from build123d import *

# Parameters (mm, degrees)
FILLET1_R           = 1
SKETCH2_R           = 10
BOSS_EXTRUDE1_DEPTH = 2.5
CUT_EXTRUDE1_DEPTH  = 10.5
BOSS_EXTRUDE2_DEPTH = 13.5


with BuildPart() as part:
    # Sketch1 → Revolve1 (revolve)
    with BuildSketch(Plane.XY):
        with BuildLine():
            Line((20, 8.32575695), (20, 0))
            Line((20, 0), (0, 0))
            Line((0, 0), (0, 12.5))
            ThreePointArc((0, 12.5), (10.215482184, 11.445315647), (20, 8.32575695))
        make_face()
    revolve(axis=Axis((0, 0, 0), (0, 1, 0)))

    # Fillet1
    fillet1_edges = [part.edges().sort_by_distance(p)[0] for p in [
        (-20, 8.32575695, 0),
    ]]
    fillet(fillet1_edges, radius=FILLET1_R)

    # Sketch2 → Boss-Extrude1 (add)
    with BuildSketch(Plane.XZ):
        Circle(SKETCH2_R)
    extrude(amount=BOSS_EXTRUDE1_DEPTH)

    # Sketch3 → Cut-Extrude1 (cut)
    with BuildSketch(Plane(origin=(0, 8, 0), x_dir=(-1, 0, 0), z_dir=(0, -1, 0))):
        with BuildLine():
            Line((7.5, 8), (7.5, -8))
            ThreePointArc((7.5, -8), (10.299205094, -11.811908762), (14.774238712, -10.282114106))
            ThreePointArc((14.774238712, -10.282114106), (18, 0), (14.774238712, 10.282114106))
            ThreePointArc((14.774238712, 10.282114106), (10.299205094, 11.811908762), (7.5, 8))
        make_face()
        with BuildLine():
            Line((-7.5, 8), (-7.5, -8))
            ThreePointArc((-7.5, -8), (-10.299205094, -11.811908762), (-14.774238712, -10.282114106))
            ThreePointArc((-14.774238712, -10.282114106), (-18, 0), (-14.774238712, 10.282114106))
            ThreePointArc((-14.774238712, 10.282114106), (-10.299205094, 11.811908762), (-7.5, 8))
        make_face()
    extrude(amount=-CUT_EXTRUDE1_DEPTH, mode=Mode.SUBTRACT)

    # Sketch5 → Boss-Extrude2 (add)
    with BuildSketch(Plane.XZ):
        Polygon((2, -12), (0, -15.464101615), (-2, -12), align=None)
        Polygon((2, 12), (0, 15.464101615), (-2, 12), align=None)
    extrude(amount=-BOSS_EXTRUDE2_DEPTH)

    # Sketch4 → Cut-Revolve3 (revolve, cut)
    with BuildSketch(Plane(origin=(0, 0, 0), x_dir=(0, 0, -1), z_dir=(1, 0, 0)), mode=Mode.PRIVATE) as cut_revolve3_sk:
        with BuildLine():
            Line((0, 17.5), (0, 13.5))
            ThreePointArc((0, 13.5), (9.805586606, 12.548481209), (19.245283019, 9.729430248))
            ThreePointArc((19.245283019, 9.729430248), (21.85213452, 10.826847786), (20.754716981, 13.433699287))
            ThreePointArc((20.754716981, 13.433699287), (10.574652222, 16.473852284), (0, 17.5))
        make_face()
    revolve(cut_revolve3_sk.sketch.rotate(Axis((0, 0, 0), (0, 1, 0)), 270), axis=Axis((0, 0, 0), (0, 1, 0)), mode=Mode.SUBTRACT)


solid = part.part
For this review, take the finished solid that the model builds, in its own axes (mm). A direction names the side the tool comes from. Round coordinates to 2 decimals unless told otherwise and drop trailing zeros. Loops run counter-clockwise (first coordinate to the right, second up) from the corner with the lowest first, then second, coordinate; pieces in that order, holes last. Notation, with made-up numbers: (76.25, 8) - (135.25, 8) arc R24 ccw to (135.25, 45) - close; hole circle Ø2 at (36.25, -38.75). An arc over 180 degrees is marked (long way). Put each result on its own line as item: value. Start each with the question number.
1. Insertion check: P1, Ø4.5, axis at y = 11, z = -1.5, coming from the +X side; P2, Ø5, axis at x = 12.5, z = -1, coming from the +Y side; P3, Ø5, axis at x = 10, y = 1.5, coming from the +Z side. Each pin has a flat end and moves straight along its axis. Give the tip position at first contact, or say it passes through.
2. Mouldability with a two-part tool opening along X and no side actions: class faces 5 (the cylindrical face through (19.076, 3.78, -6.007)), 6 (the cylindrical face through (-18, 8.6, 0.2)), 7 (the cylindrical face through (18, 8.6, 0.2)), 8 (the flat face through (1.014, 11.024, 13.708)) as +X half, -X half, draft (parallel to the pull), parting line (faces both ways), or undercut.
3. For probe 1 along Z at (x, y) = (-16, 8.25); probe 2 along Y at (x, z) = (16, -1); probe 3 along Y at (x, z) = (-4, -11.5), list the stretches that pass through material, from the lowest coordinate up. Write a range as [from, to].
4. For faces 1 (the flat face through (1.014, 11.024, -13.708)), 2 (the flat face through (-0.986, 11.024, 13.756)), 3 (the flat face through (7.5, 10, 0)), 4 (the cylindrical face through (-2.17, -1.23, -9.76)), list the 3-axis set-ups (+Z, -Z, +X, -X, +Y, -Y) from which the entire face can be reached by the end or side of a thin tool; tool diameter is ignored.
5. Consider section A-A on y = -1.5. State the section outline as (x, z) points, plus the area to 3 significant figures.
Result sheet:
1. P1: x = 18.94
1. P2: y = 8
1. P3: z = 18.54
2. face 5: parting line
2. face 6: undercut
2. face 7: undercut
2. face 8: +X half
3. probe 1: [-11.68, -8.25], [8.25, 11.68]
3. probe 2: [0, 8]
3. probe 3: [0, 10.99]
4. face 1: -Z, +X, +Y
4. face 2: +Z, -X, +Y
4. face 3: +Y
4. face 4: -Y
5. outline: circle Ø20 at (0, 0)
5. area: 314 mm^2
